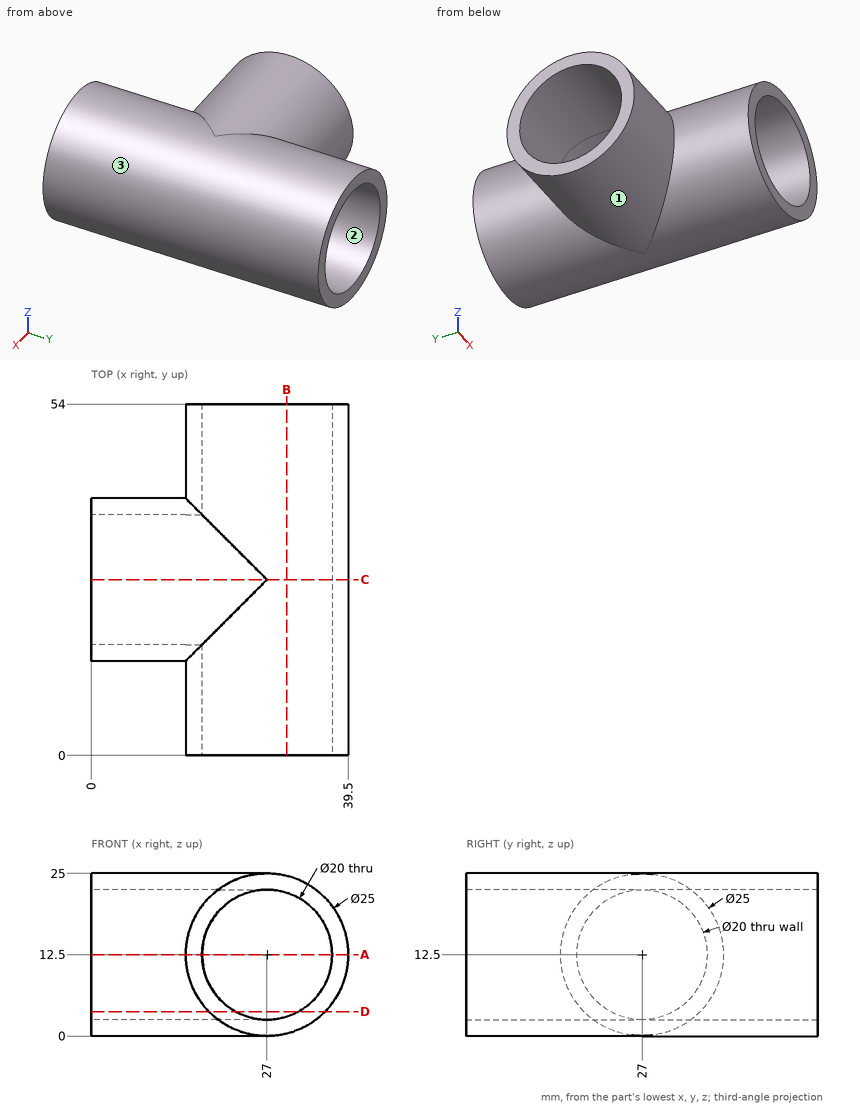
Can you work these out from the drawing? Everything is in mm from the part's minimum corner. Round coordinates to 2 decimals unless told otherwise and drop trailing zeros. Loops run counter-clockwise (first coordinate to the right, second up) from the corner with the lowest first, then second, coordinate; pieces in that order, holes last. Notation, with made-up numbers: (-37, -29) - (-2, -29) arc R24 ccw to (-2, 1) - close; hole circle Ø4 at (6, -34.75). An arc over 180 degrees is marked (long way). Answer in a Markdown table with one row per item. Add a question column.
(1) If we mould it in two halves opening along X, with no side actions, what happens to the marked faces 1, 2 and 3? For each: pulls with the +X half, pulls with the -X half, needs draft (parallel to the pull), parting line crosses it, or undercut.
(2) If we section it at D-D (z = 3.75): Please give me the cut outline in (x, y).
(3) If we section it at A-A (z = 12.5): Please give me the cut outline in (x, y), plus the area to 4 significant figures.
(4) If we section it at C-C (y = 27): Please give me the cut outline in (x, z), plus the area to 3 significant figures.
(5) I'm going to push flat-ended pins straight in: pin 1 (12 mm diameter, centred on y = 27, z = 12.5, fed in from -X); pin 2 (3 mm diameter, centred on x = 7.5, z = 13, fed in from +Y); pin 3 (2 mm diameter, centred on y = 19, z = 12.5, fed in from -X). Where does each tip first touch, or does it pass through?
(6) If we section it at B-B (x = 30): Please give me the cut outline in (y, z).
(7) I need wall thicknesses on line 1 along Y through (x, z) = (11.5, 12.5); line 2 along Z through (x, y) = (21.5, 27). Which ranges of each line are inside material? Lowest first, please.
Model answer:
| question | item | result |
|---|---|---|
| 1 | face 1 | needs draft |
| 1 | face 2 | undercut |
| 1 | face 3 | parting line crosses it |
| 2 | outline | (0, 18.07) - (18.07, 18.07) - (18.07, 0) - (22.16, 0) - (22.16, 22.16) - (0, 22.16) - close; (0, 31.84) - (22.16, 31.84) - (22.16, 54) - (18.07, 54) - (18.07, 35.93) - (0, 35.93) - close; (31.84, 0) - (35.93, 0) - (35.93, 54) - (31.84, 54) - close |
| 3 | outline | (0, 14.5) - (14.5, 14.5) - (14.5, 0) - (17, 0) - (17, 17) - (0, 17) - close; (0, 37) - (17, 37) - (17, 54) - (14.5, 54) - (14.5, 39.5) - (0, 39.5) - close; (37, 0) - (39.5, 0) - (39.5, 54) - (37, 54) - close |
| 3 | area | 292.5 mm² |
| 4 | outline | (0, 0) - (27, 0) arc R12.5 ccw to (27, 25) - (0, 25) - (0, 22.5) - (27, 22.5) arc R10 cw to (27, 2.5) - (0, 2.5) - close |
| 4 | area | 223 mm² |
| 5 | pin 1 | stops at x = 35 |
| 5 | pin 2 | stops at y = 39.5 |
| 5 | pin 3 | stops at x = 36.95 |
| 6 | outline | (0, 0.37) - (54, 0.37) - (54, 2.96) - (0, 2.96) - close; (0, 22.04) - (54, 22.04) - (54, 24.63) - (0, 24.63) - close |
| 7 | line 1 | y = 14.5 to 17, 37 to 39.5 |
| 7 | line 2 | z = 0 to 2.5, 22.5 to 25 |
